Part model, mm, in its own coordinate system. Coordinates: 2 decimals unless noted, no trailing zeros. Order: outer loops, then holes, each group sorted by start corner. A loop starts at its lowest first (then second) coordinate and runs counter-clockwise, first axis right, second up.
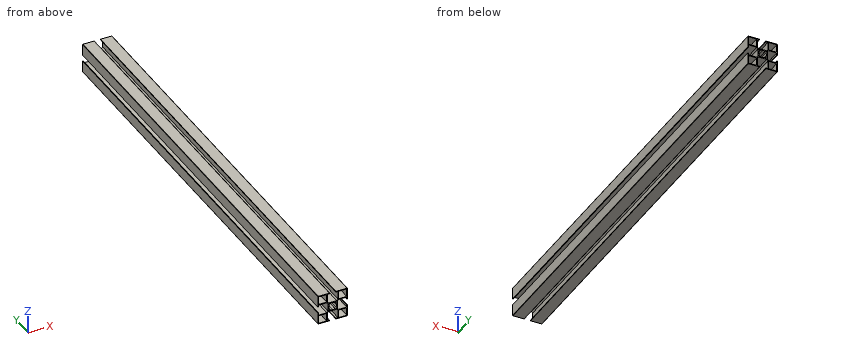
from build123d import *

# Parameters (mm, degrees)
SKETCH1_W               = 10.85
SKETCH1_H               = 10.85
BOSS_EXTRUDE1_DEPTH     = 620
MIRROR2_COPY_1_SKETCH_W = 10.85
MIRROR2_COPY_1_SKETCH_H = 10.85
MIRROR2_COPY_1_DEPTH    = 620


with BuildPart() as part:
    # Sketch1 → Boss-Extrude1 (new body)
    with BuildSketch(Plane(origin=(0, 0, 0), x_dir=(1, 0, 0), z_dir=(0, 1, 0))):
        with BuildLine():
            Line((-4.3, 20), (-19.5, 20))
            ThreePointArc((-19.5, 20), (-19.853553391, 19.853553391), (-20, 19.5))
            Line((-20, 19.5), (-20, 4.3))
            Line((-20, 4.3), (-19.05, 4.3))
            Line((-19.05, 4.3), (-19.05, 7.25))
            Line((-19.05, 7.25), (-7.921751442, 7.25))
            Line((-7.921751442, 7.25), (-6.2, 5.528248558))
            Line((-6.2, 5.528248558), (-6.2, 0))
            Line((-6.2, 0), (-5.3, 0))
            ThreePointArc((-5.3, 0), (-5.066731596, 1.555066215), (-4.387460025, 2.973246463))
            Line((-4.387460025, 2.973246463), (-5.091168825, 3.676955262))
            ThreePointArc((-5.091168825, 3.676955262), (-5.091168825, 5.091168825), (-3.676955262, 5.091168825))
            Line((-3.676955262, 5.091168825), (-2.973246463, 4.387460025))
            ThreePointArc((-2.973246463, 4.387460025), (-1.555066215, 5.066731596), (0, 5.3))
            Line((0, 5.3), (0, 6.2))
            Line((0, 6.2), (-5.528248558, 6.2))
            Line((-5.528248558, 6.2), (-7.25, 7.921751442))
            Line((-7.25, 7.921751442), (-7.25, 19.05))
            Line((-7.25, 19.05), (-4.3, 19.05))
            Line((-4.3, 19.05), (-4.3, 20))
        make_face()
        with Locations((-13.625, 13.625)):
            Rectangle(SKETCH1_W, SKETCH1_H, mode=Mode.SUBTRACT)
    boss_extrude1 = extrude(amount=BOSS_EXTRUDE1_DEPTH)

    # Mirror1: Boss-Extrude1 across plane
    add(boss_extrude1.mirror(Plane(origin=(0, 0, 0), x_dir=(0, 0, 1), z_dir=(1, 0, 0))))

    # Mirror2: Boss-Extrude1 across plane
    add(boss_extrude1.mirror(Plane.XY))

    # Mirror2 copy 1 sketch → Mirror2 copy 1 (add)
    with BuildSketch(Plane(origin=(0, 0, 0), x_dir=(-1, 0, 0), z_dir=(0, 1, 0))):
        with BuildLine():
            Line((-4.3, 20), (-19.5, 20))
            ThreePointArc((-19.5, 20), (-19.853553391, 19.853553391), (-20, 19.5))
            Line((-20, 19.5), (-20, 4.3))
            Line((-20, 4.3), (-19.05, 4.3))
            Line((-19.05, 4.3), (-19.05, 7.25))
            Line((-19.05, 7.25), (-7.921751442, 7.25))
            Line((-7.921751442, 7.25), (-6.2, 5.528248558))
            Line((-6.2, 5.528248558), (-6.2, 0))
            Line((-6.2, 0), (-5.3, 0))
            ThreePointArc((-5.3, 0), (-5.066731596, 1.555066215), (-4.387460025, 2.973246463))
            Line((-4.387460025, 2.973246463), (-5.091168825, 3.676955262))
            ThreePointArc((-5.091168825, 3.676955262), (-5.091168825, 5.091168825), (-3.676955262, 5.091168825))
            Line((-3.676955262, 5.091168825), (-2.973246463, 4.387460025))
            ThreePointArc((-2.973246463, 4.387460025), (-1.555066215, 5.066731596), (0, 5.3))
            Line((0, 5.3), (0, 6.2))
            Line((0, 6.2), (-5.528248558, 6.2))
            Line((-5.528248558, 6.2), (-7.25, 7.921751442))
            Line((-7.25, 7.921751442), (-7.25, 19.05))
            Line((-7.25, 19.05), (-4.3, 19.05))
            Line((-4.3, 19.05), (-4.3, 20))
        make_face()
        with Locations((-13.625, 13.625)):
            Rectangle(MIRROR2_COPY_1_SKETCH_W, MIRROR2_COPY_1_SKETCH_H, mode=Mode.SUBTRACT)
    extrude(amount=MIRROR2_COPY_1_DEPTH)


solid = part.part
Q1. Cut at A-A on z = 14. Write the cut outline in (x, y).
Results list:
outline: (-20, 0) - (-19.05, 0) - (-19.05, 620) - (-20, 620) - close; (-8.2, 0) - (-7.25, 0) - (-7.25, 620) - (-8.2, 620) - close; (7.25, 0) - (8.2, 0) - (8.2, 620) - (7.25, 620) - close; (19.05, 0) - (20, 0) - (20, 620) - (19.05, 620) - close
Q2. Wall check: line 1 along X through (y, z) = (267.5, -9); line 2 along Z through (x, y) = (4, 156). Give the ranges that are in metal, low to high.
Results list:
line 1: x = -20 to -19.05, -8.2 to -7.25, 7.25 to 8.2, 19.05 to 20
line 2: z = -6.2 to -5.31, 5.31 to 6.2
Q3. Cut at B-B on y = 74. Count the separate pieces of the cut face and the enclosed holes in it, and give its area (3 significant figures).
Results list:
separate pieces: 1
enclosed holes: 5
area: 261 mm2
